Design review of the part built by this model. Coordinates are the model's own, in mm. A direction names the side the tool comes from. Coordinates: 2 decimals unless noted, no trailing zeros. Loops run counter-clockwise (first coordinate to the right, second up) from the corner with the lowest first, then second, coordinate; pieces in that order, holes last. Notation, with made-up numbers: M 4.25,74 L 21.25,74 A31 cw 21.25,111 Z; hole C 22.5,-35 d4. An arc over 180 degrees is marked long. Answer as a JSON object with one key per item and string values. Group by question number.
1. To check wall thickness, follow probe 1 along Y at (x, z) = (61, 32); probe 2 along X at (y, z) = (263, 3); probe 3 along Y at (x, z) = (28, 23.5). State the ranges of each line that lie inside material, in increasing order.
2. Consider section C-C (y = 91). State the section outline as (x, z) points, then the cut area to 3 significant figures.
3. Draft analysis for pull direction Y (two halves, no side actions). For faces 4 (the flat face through (1, 270, 32)), 5 (the flat face through (1, 0, -1)), 6 (the flat face through (61, 250, -23)), state which applies: +Y half, -Y half, draft (parallel to the pull), parting line (faces both ways), or undercut.
4. Consider section A-A (z = 0). State the section outline as (x, y) points.
5. Insertion check: pin 1 (3 mm diameter, centred on x = -1, y = 97.5, fed in from -Z); pin 2 (1 mm diameter, centred on y = 123.5, z = 42.5, fed in from -X); pin 3 (3 mm diameter, centred on x = 50, z = 13, fed in from +Y); pin 4 (1 mm diameter, centred on x = -59.5, y = 142, fed in from +Z). Each pin has a flat end and moves straight along its axis. Give the tip position at first contact, or say it passes through.
6. Machinability: for faces 1 (the cylindrical face through (19.52, 254.93, 62)), 2 (the cylindrical face through (7.509, 279.367, 23.846)), 3 (the cylindrical face through (-45.636, 264.437, -59.517)), which of the approach directions +Z, -Z, +X, -X, +Y, -Y give a long, thin tool a straight path to every point of the face, cutting with its end or side? Answer none if there is none.
7. Consider section B-B (x = 0). State the section outline as (y, z) points.
from build123d import *

# Parameters (mm, degrees)
SKETCH1_R           = 75
BOSS_EXTRUDE1_DEPTH = 250
SKETCH2_R           = 65
BOSS_EXTRUDE2_DEPTH = 10
SKETCH3_R           = 75
BOSS_EXTRUDE3_DEPTH = 10
SKETCH4_R           = 25
BOSS_EXTRUDE4_DEPTH = 20
FILLET1_R           = 1
CHAMFER1_SIZE       = 1


with BuildPart() as part:
    # Sketch1 → Boss-Extrude1 (new body)
    with BuildSketch(Plane(origin=(0, 0, 0), x_dir=(1, 0, 0), z_dir=(0, 1, 0))):
        with Locations(Location((0, 0, 0), (0, 0, 270))):
            Circle(SKETCH1_R)
    extrude(amount=BOSS_EXTRUDE1_DEPTH)

    # Sketch2 → Boss-Extrude2 (add)
    with BuildSketch(Plane(origin=(0, 250, 0), x_dir=(1, 0, 0), z_dir=(0, 1, 0))):
        with Locations(Location((0, 0, 0), (0, 0, 270))):
            Circle(SKETCH2_R)
    extrude(amount=BOSS_EXTRUDE2_DEPTH)

    # Sketch3 → Boss-Extrude3 (add)
    with BuildSketch(Plane(origin=(0, 260, 0), x_dir=(1, 0, 0), z_dir=(0, 1, 0))):
        with Locations(Location((0, 0, 0), (0, 0, 270))):
            Circle(SKETCH3_R)
    extrude(amount=BOSS_EXTRUDE3_DEPTH)

    # Sketch4 → Boss-Extrude4 (add)
    with BuildSketch(Plane(origin=(0, 270, 0), x_dir=(1, 0, 0), z_dir=(0, 1, 0))):
        with Locations(Location((0, 0, 0), (0, 0, 270))):
            Circle(SKETCH4_R)
    extrude(amount=BOSS_EXTRUDE4_DEPTH)

    # Fillet1
    fillet1_edges = [part.edges().sort_by_distance(p)[0] for p in [
        (0, 290, -25),
    ]]
    fillet(fillet1_edges, radius=FILLET1_R)

    # Chamfer1
    chamfer1_edges = [part.edges().sort_by_distance(p)[0] for p in [
        (0, 270, -75),
    ]]
    chamfer(chamfer1_edges, length=CHAMFER1_SIZE)


solid = part.part
Findings below:
{
 "1": {"probe 1": "y = 0 to 250, 260 to 270", "probe 2": "x = -74.94 to 74.94", "probe 3": "y = 0 to 270"},
 "2": {"outline": "C 0,0 d150", "area": "17,700 mm^2"},
 "3": {"face 4": "+Y half", "face 5": "-Y half", "face 6": "undercut"},
 "4": {"outline": "M -75,0 L 75,0 L 75,250 L 65,250 L 65,260 L 75,260 L 75,269 L 74,270 L 25,270 L 25,289 A1 ccw 24,290 L -24,290 A1 ccw -25,289 L -25,270 L -74,270 L -75,269 L -75,260 L -65,260 L -65,250 L -75,250 Z"},
 "5": {"pin 1": "stops at z = -75", "pin 2": "stops at x = -62.14", "pin 3": "stops at y = 270", "pin 4": "stops at z = 46.3"},
 "6": {"face 1": "none", "face 2": "+Y", "face 3": "+Y, -Y"},
 "7": {"outline": "M 0,-75 L 250,-75 L 250,-65 L 260,-65 L 260,-75 L 269,-75 L 270,-74 L 270,-25 L 289,-25 A1 ccw 290,-24 L 290,24 A1 ccw 289,25 L 270,25 L 270,74 L 269,75 L 260,75 L 260,65 L 250,65 L 250,75 L 0,75 Z"}
}
